```python
from build123d import *

# Parameters (mm, degrees)
SLEEVE_PROFILE_65_32_R   = 32.5
SLEEVE_PROFILE_65_32_R_2 = 16
SLEEVE_65X100_DEPTH      = 50
BRACKET_WEB_DEPTH        = 32.5
SIDE_RAILS_DEPTH         = 65
LUG_START                = -255
LUG_HOLE_PROFILE_R       = 16
LUG_HOLE_THROUGH_DEPTH   = 255


with BuildPart() as part:
    # Sleeve Profile Ø65-Ø32 → Sleeve Ø65x100 (new, symmetric)
    with BuildSketch(Plane(origin=(0, 0, 0), x_dir=(0, 0, -1), z_dir=(1, 0, 0))):
        Circle(SLEEVE_PROFILE_65_32_R)
        Circle(SLEEVE_PROFILE_65_32_R_2, mode=Mode.SUBTRACT)
    extrude(amount=SLEEVE_65X100_DEPTH, both=True)



with BuildPart() as body_2:
    # Bracket Web Profile → Bracket Web (new, symmetric)
    with BuildSketch(Plane.XY):
        with BuildLine():
            Line((0, -32.5), (-28.5, -32.5))
            ThreePointArc((-28.5, -32.5), (-24.257359313, -34.257359313), (-22.5, -38.5))
            Line((-22.5, -38.5), (-22.5, -52))
            ThreePointArc((-22.5, -52), (0, -74.5), (22.5, -52))
            Line((22.5, -52), (22.5, -38.5))
            ThreePointArc((22.5, -38.5), (24.257359313, -34.257359313), (28.5, -32.5))
            Line((28.5, -32.5), (0, -32.5))
        make_face()
        with BuildLine():
            Line((-5, -35.543560763), (0, -35.543560763))
            Line((0, -35.543560763), (5, -35.543560763))
            Line((5, -35.543560763), (5, -40.543560763))
            ThreePointArc((5, -40.543560763), (0, -64.5), (-5, -40.543560763))
            Line((-5, -40.543560763), (-5, -35.543560763))
        make_face(mode=Mode.SUBTRACT)
    extrude(amount=BRACKET_WEB_DEPTH, both=True)


with BuildPart() as part_1:
    add(part.part)

    add(body_2.part)  # Side Rails merges body 2
    # Side Rail Profile → Side Rails (add)
    # profile 1 of 9: a face of its own
    with BuildSketch(Plane.XY.offset(32.5)):
        with BuildLine():
            Line((-22.5, -32.5), (-28.5, -32.5))
            ThreePointArc((-28.5, -32.5), (-24.257359313, -34.257359313), (-22.5, -38.5))
            Line((-22.5, -38.5), (-22.5, -32.5))
        make_face()
    # profile 2 of 9: a face of its own
    with BuildSketch(Plane.XY.offset(32.5)):
        with BuildLine():
            Line((-23.44711749, -7.891120858), (-28.5, 0))
            Line((-28.5, 0), (-28.5, -32.5))
            Line((-28.5, -32.5), (-22.5, -32.5))
            Line((-22.5, -32.5), (-22.5, -11.126608201))
            ThreePointArc((-22.5, -11.126608201), (-22.741645415, -9.440977022), (-23.44711749, -7.891120858))
        make_face()
    # profile 3 of 9: a face of its own
    with BuildSketch(Plane.XY.offset(32.5)):
        with BuildLine():
            Line((28.5, 0), (-28.5, 0))
            Line((-28.5, 0), (-23.44711749, -7.891120858))
            ThreePointArc((-23.44711749, -7.891120858), (-22.741645415, -9.440977022), (-22.5, -11.126608201))
            Line((-22.5, -11.126608201), (-22.5, -32.5))
            Line((-22.5, -32.5), (-11.22497216, -32.5))
            ThreePointArc((-11.22497216, -32.5), (0, -29.5), (11.22497216, -32.5))
            Line((11.22497216, -32.5), (22.5, -32.5))
            Line((22.5, -32.5), (22.5, -11.126608201))
            ThreePointArc((22.5, -11.126608201), (22.741645415, -9.440977022), (23.44711749, -7.891120858))
            Line((23.44711749, -7.891120858), (28.5, 0))
        make_face()
    # profile 4 of 9: a face of its own
    with BuildSketch(Plane.XY.offset(32.5)):
        with BuildLine():
            Line((28.5, -32.5), (28.5, 0))
            Line((28.5, 0), (23.44711749, -7.891120858))
            ThreePointArc((23.44711749, -7.891120858), (22.741645415, -9.440977022), (22.5, -11.126608201))
            Line((22.5, -11.126608201), (22.5, -32.5))
            Line((22.5, -32.5), (28.5, -32.5))
        make_face()
    # profile 5 of 9: a face of its own
    with BuildSketch(Plane.XY.offset(32.5)):
        with BuildLine():
            Line((22.5, -52), (22.5, -38.5))
            Line((22.5, -38.5), (22.5, -32.5))
            Line((22.5, -32.5), (11.22497216, -32.5))
            ThreePointArc((11.22497216, -32.5), (19.47834533, -40.737493032), (22.5, -52))
        make_face()
    # profile 6 of 9: a face of its own
    with BuildSketch(Plane.XY.offset(32.5)):
        with BuildLine():
            ThreePointArc((22.5, -38.5), (24.257359313, -34.257359313), (28.5, -32.5))
            Line((28.5, -32.5), (22.5, -32.5))
            Line((22.5, -32.5), (22.5, -38.5))
        make_face()
    # profile 7 of 9: a face of its own
    with BuildSketch(Plane.XY.offset(32.5)):
        with BuildLine():
            Line((-22.5, -32.5), (-22.5, -38.5))
            Line((-22.5, -38.5), (-22.5, -52))
            ThreePointArc((-22.5, -52), (-19.47834533, -40.737493032), (-11.22497216, -32.5))
            Line((-11.22497216, -32.5), (-22.5, -32.5))
        make_face()
    # profile 8 of 9: a face of its own
    with BuildSketch(Plane.XY.offset(32.5)):
        with BuildLine():
            ThreePointArc((-11.22497216, -32.5), (-19.47834533, -40.737493032), (-22.5, -52))
            ThreePointArc((-22.5, -52), (0, -74.5), (22.5, -52))
            ThreePointArc((22.5, -52), (19.47834533, -40.737493032), (11.22497216, -32.5))
            Line((11.22497216, -32.5), (-11.22497216, -32.5))
        make_face()
        with BuildLine():
            ThreePointArc((5, -40.543560763), (0, -64.5), (-5, -40.543560763))
            Line((-5, -40.543560763), (-5, -35.543560763))
            Line((-5, -35.543560763), (5, -35.543560763))
            Line((5, -35.543560763), (5, -40.543560763))
        make_face(mode=Mode.SUBTRACT)
    # profile 9 of 9: a face of its own
    with BuildSketch(Plane.XY.offset(32.5)):
        with BuildLine():
            ThreePointArc((11.22497216, -32.5), (0, -29.5), (-11.22497216, -32.5))
            Line((-11.22497216, -32.5), (11.22497216, -32.5))
        make_face()
    extrude(amount=-SIDE_RAILS_DEPTH)

    # Lug Hole Profile → Lug Hole Through (cut)
    with BuildSketch(Plane(origin=(50, 0, 0), x_dir=(0, 0, -1), z_dir=(1, 0, 0)).offset(LUG_START)):
        Circle(LUG_HOLE_PROFILE_R)
    extrude(amount=LUG_HOLE_THROUGH_DEPTH, mode=Mode.SUBTRACT)


solid = part_1.part
```
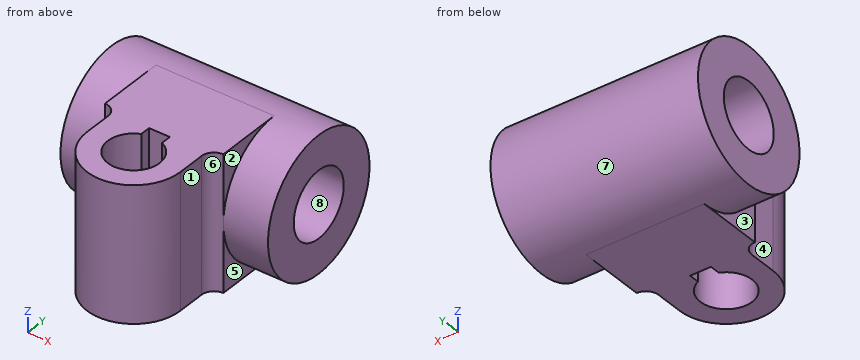
CAD build for the part. Positions are in the model's coordinates, mm. Face numbers are marked on the shaded views. A direction names the side the tool comes from. Give positions to 0.01 mm unless a question says otherwise; leave off trailing zeros. Order: outer loops, then holes, each group sorted by start corner. A loop starts at its lowest first (then second) coordinate and runs counter-clockwise, first axis right, second up.
(1) Saw through at D-D, the plane z = -22. Give the cut face in (x, y).
(2) Drill centre lines: L1, parallel to Y at x = 0, z = 0; L2, parallel to Y at x = -6, z = 14; L3, parallel to X at y = -52, z = 8. Where is each one in solid material? Low to high.
(3) Mould opens along Z. For the marked faces 6, 7 and 8 say: released by +Z, released by -Z, zero draft, split by the parting line, or undercut.
(4) Flat gauge pins, fed straight in: pin 1 (8 mm diameter, centred on x = 0, z = -7.5, fed in from -Y); pin 2 (2 mm diameter, centred on x = 24.5, z = -20.5, fed in from +Y); pin 3 (6 mm diameter, centred on y = -49.5, z = 5, fed in from +X); pin 4 (22.5 mm diameter, centred on x = 0, y = -52, fed in from +Z). Where does each tip first touch, or does it go through?
(5) Saw through at C-C, the plane y = -58. Give the cut face in (x, z), then the cut area to 3 significant figures.
(6) Saw through at B-B, the plane z = 5. Give the cut face in (x, y), then the cut area to 3 significant figures.
(7) Saw through at A-A, the plane x = 0. Give the cut face in (y, z).
(8) Tool access for the marked faces 1, 2, 3, 4 and 5: list every direction of +Z, -Z, +X, -X, +Y, -Y with a clear straight run to the whole face (end or side of a thin tool).
Results found:
1. outline: (-50, -23.92) - (-28.5, -23.92) - (-28.5, -32.5) arc R6 cw to (-22.5, -38.5) - (-22.5, -52) arc R22.5 ccw to (22.5, -52) - (22.5, -38.5) arc R6 cw to (28.5, -32.5) - (28.5, -23.92) - (50, -23.92) - (50, 23.92) - (-50, 23.92) - close; hole (-5, -40.54) arc R12.5 ccw (long way) to (5, -40.54) - (5, -35.54) - (-5, -35.54) - close
2. L1: y = -74.5 to -64.5, -35.54 to -16, 16 to 32.5
2. L2: y = -73.69 to -62.97, -41.03 to -7.75, 7.75 to 29.33
2. L3: x = -22.5 to -12.5, 12.5 to 22.5
3. face 6: zero draft
3. face 7: split by the parting line
3. face 8: undercut
4. pin 1: stops at y = -74.5
4. pin 2: stops at y = 26
4. pin 3: stops at x = 22.5
4. pin 4: passes through
5. outline: (-21.69, -32.5) - (-10.97, -32.5) - (-10.97, 32.5) - (-21.69, 32.5) - close; (10.97, -32.5) - (21.69, -32.5) - (21.69, 32.5) - (10.97, 32.5) - close
5. area: 1,390 mm2
6. outline: (-50, -32.11) - (-28.5, -32.11) - (-28.5, -32.5) arc R6 cw to (-22.5, -38.5) - (-22.5, -52) arc R22.5 ccw to (22.5, -52) - (22.5, -38.5) arc R6 cw to (28.5, -32.5) - (28.5, -32.11) - (50, -32.11) - (50, -15.2) - (-50, -15.2) - close; (-50, 15.2) - (50, 15.2) - (50, 32.11) - (-50, 32.11) - close; hole (-5, -40.54) arc R12.5 ccw (long way) to (5, -40.54) - (5, -35.54) - (-5, -35.54) - close
6. area: 4,560 mm2
7. outline: (-74.5, -32.5) - (-64.5, -32.5) - (-64.5, 32.5) - (-74.5, 32.5) - close; (-35.54, -32.5) - (0, -32.5) arc R32.5 ccw to (0, 32.5) - (-35.54, 32.5) - close; hole circle Ø32 at (0, 0)
8. face 1: +Z, -Z, +X, -Y
8. face 2: +Z, +X, -Y
8. face 3: -Z, -X, -Y
8. face 4: +Z, -Z, -X, -Y
8. face 5: -Z, +X, -Y
